For this review, take the finished solid that the model builds, in its own axes (mm). A direction names the side the tool comes from. Round coordinates to 2 decimals unless told otherwise and drop trailing zeros. Write each loop counter-clockwise with the first axis right and the second up, starting at its lowest first coordinate (ties: lowest second). Pieces come first, ordered by that corner, then holes.
from build123d import *

# Parameters (mm, degrees)
SKETCH_1_W          = 45
SKETCH_1_H          = 15
EXTRUDE_1_DEPTH     = 3.5
CUT_EXTRUDE_1_DEPTH = 5
SKETCH_5_R          = 5
EXTRUDE_2_DEPTH     = 290


with BuildPart() as part:
    # 草图1 → 凸台-拉伸1 (new, symmetric)
    with BuildSketch(Plane(origin=(0, 0, 0), x_dir=(1, 0, 0), z_dir=(0, 1, 0))):
        with Locations((22.5, 0)):
            Rectangle(SKETCH_1_W, SKETCH_1_H)
    extrude(amount=EXTRUDE_1_DEPTH, both=True)

    # 草图2 → 旋转1 (revolve)
    with BuildSketch(Plane.XY, mode=Mode.PRIVATE) as revolve_1_sk:
        Polygon((45, 3.5), (45, 0), (100, 0), (100, 5), (50, 5), (45, 5), align=None)
    revolve(revolve_1_sk.sketch.rotate(Axis((3.468083249, 0, 0), (1, 0, 0)), 90), axis=Axis((3.468083249, 0, 0), (1, 0, 0)))

    # 草图3 → 切除-拉伸1 (cut, symmetric)
    with BuildSketch(Plane.XY):
        with BuildLine():
            Line((50, -5), (50, -7.872092098))
            Line((50, -7.872092098), (45, -7.872092098))
            Line((45, -7.872092098), (45, -3.5))
            ThreePointArc((45, -3.5), (47.610076627, -3.883077909), (50, -5))
        make_face()
        with BuildLine():
            Line((45, 3.5), (45, 6.877663773))
            Line((45, 6.877663773), (50, 6.877663773))
            Line((50, 6.877663773), (50, 5))
            ThreePointArc((50, 5), (47.610076627, 3.883077909), (45, 3.5))
        make_face()
    extrude(amount=CUT_EXTRUDE_1_DEPTH, both=True, mode=Mode.SUBTRACT)

    # 草图4 → 切除-旋转1 (revolve, cut)
    with BuildSketch(Plane(origin=(0, 0, 0), x_dir=(1, 0, 0), z_dir=(0, 1, 0))):
        with BuildLine():
            Line((40, 11.25), (45, 11.25))
            Line((45, 11.25), (45, 5))
            ThreePointArc((45, 5), (42.204915028, 5.659830056), (40, 7.5))
            ThreePointArc((40, 7.5), (39.341282089, 8.596434171), (38.919571519, 9.804009168))
            Line((38.919571519, 9.804009168), (40, 11.25))
        make_face()
    revolve(axis=Axis((45, 0, 0), (-1, 0, 0)), mode=Mode.SUBTRACT)

    # 草图5 → 凸台-拉伸2 (add)
    with BuildSketch(Plane(origin=(100, 0, 0), x_dir=(0, 0, -1), z_dir=(1, 0, 0))):
        with Locations(Location((0, 0, 0), (0, 0, 135.572995999))):
            Circle(SKETCH_5_R)
    extrude(amount=EXTRUDE_2_DEPTH)

    # 镜向1: part across plane


with BuildPart() as part_1:
    add(part.part)
    add(part.part.mirror(Plane(origin=(390, 0, 0), x_dir=(0, 0, 1), z_dir=(1, 0, 0))))


solid = part_1.part
(1) For line 1 along Y through (x, z) = (72.5, -3.5); line 2 along Z through (x, y) = (627, -0.5); line 3 along X through (y, z) = (-3, -5.5), list the stretches that pass through material, from the lowest coordinate up.
Geometry check:
line 1: y = -3.57 to 3.57
line 2: z = -4.97 to 4.97
line 3: x = 0 to 41.23, 738.77 to 780
(2) We need section A-A, the plane z = 0. Give the boundary of the cut face in (x, y).
Geometry check:
outline: (0, -3.5) - (45, -3.5) arc R9.08 cw to (50, -5) - (730, -5) arc R9.08 cw to (735, -3.5) - (780, -3.5) - (780, 3.5) - (735, 3.5) arc R9.08 cw to (730, 5) - (50, 5) arc R9.08 cw to (45, 3.5) - (0, 3.5) - close
(3) For pin 1 Ø3 at (x, y) = (537.5, -0.5) entering from +Z; pin 2 Ø1 at (x, y) = (551.5, -4) entering from +Z; pin 3 Ø2 at (x, y) = (456, -3.5) entering from +Z, all flat-tipped, find the tip position at first contact; note any pin that passes through.
Geometry check:
pin 1: stops at z = 5
pin 2: stops at z = 3.57
pin 3: stops at z = 4.33
(4) We need section B-B, the plane x = 311. Give the boundary of the cut face in (y, z).
Geometry check:
outline: circle Ø10 at (0, 0)
(5) For faces 1 (the face through (22, -3.5, 0)), 2 (the face through (758, -3.5, 0)), 3 (the face through (22, 3.5, 0)), 4 (the face through (758, 3.5, 0)), list the 3-axis set-ups (+Z, -Z, +X, -X, +Y, -Y) from which the entire face can be reached by the end or side of a thin tool; tool diameter is ignored.
Geometry check:
face 1: +Z, -Z, -X, -Y
face 2: +Z, -Z, +X, -Y
face 3: +Z, -Z, -X, +Y
face 4: +Z, -Z, +X, +Y
